Build history of the part. All positions in model axes, mm. A direction names the side the tool comes from. Give positions to 0.01 mm unless a question says otherwise; leave off trailing zeros. Order: outer loops, then holes, each group sorted by start corner. A loop starts at its lowest first (then second) coordinate and runs counter-clockwise, first axis right, second up. Notation, with made-up numbers: (41.25, 6.25) - (59.25, 6.25) arc R16 ccw to (59.25, 14.25) - close; hole circle Ø3 at (-35, 79.5). An arc over 180 degrees is marked (long way). Answer in a Markdown table with one row per item.
```python
from build123d import *

# Parameters (mm, degrees)
CHAMFER1_SIZE      = 1
CHAMFER2_SIZE      = 1
SKETCH2_W          = 8.284694005
SKETCH2_H          = 60
SKETCH2_W_2        = 10.903172422
SKETCH2_H_2        = 30.692001108
CUT_EXTRUDE1_DEPTH = 10


with BuildPart() as part:
    # Sketch1 → Revolve1 (revolve)
    with BuildSketch(Plane.XY, mode=Mode.PRIVATE) as revolve1_sk:
        Polygon((-26.210699301, 0), (-26.210699301, 15.59), (-11.710699301, 15.59), (-9.710699301, 12.12), (-9.710699301, 8), (77.639300699, 8), (77.639300699, 0), align=None)
    revolve(revolve1_sk.sketch.rotate(Axis((-41.923036121, 0, 0), (1, 0, 0)), 90), axis=Axis((-41.923036121, 0, 0), (1, 0, 0)))

    # Chamfer1
    chamfer1_edges = [part.edges().sort_by_distance(p)[0] for p in [
        (-26.210699301, 0, -15.59),
    ]]
    chamfer(chamfer1_edges, length=CHAMFER1_SIZE)

    # Chamfer2
    chamfer2_edges = [part.edges().sort_by_distance(p)[0] for p in [
        (77.639300699, 0, -8),
    ]]
    chamfer(chamfer2_edges, length=CHAMFER2_SIZE)

    # Sketch2 → Cut-Extrude1 (cut)
    with BuildSketch(Plane.ZY.offset(26.210699301)):
        with Locations((-14.642347003, 15.254961706)):
            Rectangle(SKETCH2_W, SKETCH2_H)
        with Locations((15.951586211, 0.214629378)):
            Rectangle(SKETCH2_W_2, SKETCH2_H_2)
    extrude(amount=-CUT_EXTRUDE1_DEPTH, mode=Mode.SUBTRACT)


solid = part.part
```
1. Cut at A-A on y = 0. Write the cut outline in (x, z), and give its area (3 significant figures).
Check result:
| item | result |
|---|---|
| outline | (-26.21, -10.5) - (-16.21, -10.5) - (-16.21, -15.59) - (-11.71, -15.59) - (-9.71, -12.12) - (-9.71, -8) - (76.64, -8) - (77.64, -7) - (77.64, 7) - (76.64, 8) - (-9.71, 8) - (-9.71, 12.12) - (-11.71, 15.59) - (-16.21, 15.59) - (-16.21, 10.5) - (-26.21, 10.5) - close |
| area | 1,800 mm² |
2. Cut at D-D on x = -13. Write the cut outline in (y, z).
Check result:
| item | result |
|---|---|
| outline | circle Ø31.18 at (0, 0) |
3. Cut at B-B on z = 0. Write the cut outline in (x, y).
Check result:
| item | result |
|---|---|
| outline | (-26.21, -14.59) - (-25.21, -15.59) - (-11.71, -15.59) - (-9.71, -12.12) - (-9.71, -8) - (76.64, -8) - (77.64, -7) - (77.64, 7) - (76.64, 8) - (-9.71, 8) - (-9.71, 12.12) - (-11.71, 15.59) - (-25.21, 15.59) - (-26.21, 14.59) - close |
4. Which spindle directions (+Z, -Z, +X, -X, +Y, -Y) get a long thin tool onto all of the face, cutting with end or side? Do faces 1 (the face through (-9.711, 8, 3)), 2 (the face through (-21, 0, -10.5)), 3 (the face through (-16.211, 0, 12)). Say none if no direction does.
Check result:
| item | result |
|---|---|
| face 1 | +X |
| face 2 | -Z, -X, +Y, -Y |
| face 3 | +Z, -X, +Y, -Y |
5. Drop flat-ended pins along their axis: P1, Ø2.5, axis at y = 2.5, z = -12.5, coming from the -X side; P2, Ø1.5, axis at x = 5.5, y = 6.5, coming from the +Z side; P3, Ø11, axis at x = -22, y = -5.5, coming from the +Z side. Give the stop position or say it passes through.
Check result:
| item | result |
|---|---|
| P1 | stops at x = -16.21 |
| P2 | stops at z = 5.56 |
| P3 | stops at z = 10.5 |
6. Probe line 1 (X direction, y = -11, z = 1); line 2 (Y direction, x = 22.5, z = 0); line 3 (Z direction, x = -18, y = -0.5). List the from-to ranges inside material, lowest first.
Check result:
| item | result |
|---|---|
| line 1 | x = -26.21 to -9.71 |
| line 2 | y = -8 to 8 |
| line 3 | z = -10.5 to 10.5 |
7. Cut at C-C on x = 60.5. Write the cut outline in (y, z), and give its area (3 significant figures).
Check result:
| item | result |
|---|---|
| outline | circle Ø16 at (0, 0) |
| area | 201 mm² |
